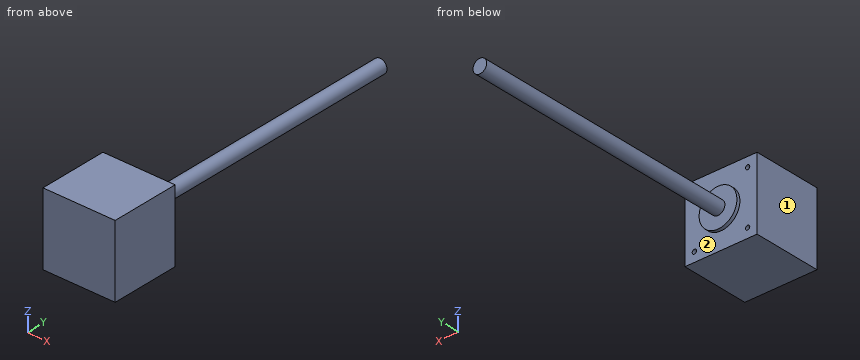
from build123d import *

# Parameters (mm, degrees)
SKETCH1_W             = 42
SKETCH1_H             = 42
BOSS_EXTRUDE1_DEPTH   = 40
SKETCH2_R             = 11
BOSS_EXTRUDE2_DEPTH   = 2
SKETCH3_R             = 4
BOSS_EXTRUDE3_DEPTH   = 159
SKETCH4_R             = 0.75
CUT_EXTRUDE1_DEPTH    = 5
M3_TAPPED_HOLE1_D     = 2.5
M3_TAPPED_HOLE1_DEPTH = 7.5
M3_TAPPED_HOLE1_TIP   = 0.751075774


with BuildPart() as part:
    # Sketch1 → Boss-Extrude1 (new body)
    with BuildSketch(Plane(origin=(0, 0, 0), x_dir=(1, 0, 0), z_dir=(0, 1, 0))):
        Rectangle(SKETCH1_W, SKETCH1_H)
    extrude(amount=BOSS_EXTRUDE1_DEPTH)

    # Sketch2 → Boss-Extrude2 (add)
    with BuildSketch(Plane(origin=(0, 40, 0), x_dir=(1, 0, 0), z_dir=(0, 1, 0))):
        with Locations(Location((0, 0, 0), (0, 0, 270))):
            Circle(SKETCH2_R)
    extrude(amount=BOSS_EXTRUDE2_DEPTH)

    # Sketch3 → Boss-Extrude3 (add)
    with BuildSketch(Plane(origin=(0, 42, 0), x_dir=(1, 0, 0), z_dir=(0, 1, 0))):
        with Locations(Location((0, 0, 0), (0, 0, 90))):
            Circle(SKETCH3_R)
    extrude(amount=BOSS_EXTRUDE3_DEPTH)

    # Sketch4 → Cut-Extrude1 (cut)
    with BuildSketch(Plane(origin=(0, 40, 0), x_dir=(1, 0, 0), z_dir=(0, 1, 0))):
        with Locations(Location((-15.5, 15.5, 0), (0, 0, 270))):
            Circle(SKETCH4_R)
        with Locations(Location((15.5, 15.5, 0), (0, 0, 270))):
            Circle(SKETCH4_R)
        with Locations(Location((15.5, -15.5, 0), (0, 0, 270))):
            Circle(SKETCH4_R)
        with Locations(Location((-15.5, -15.5, 0), (0, 0, 270))):
            Circle(SKETCH4_R)
    extrude(amount=-CUT_EXTRUDE1_DEPTH, mode=Mode.SUBTRACT)

    # M3 Tapped Hole1
    with Locations(Plane(origin=(0, 40, 0), x_dir=(1, 0, 0), z_dir=(0, 1, 0))):
        with Locations((-15.5, 15.5), (15.5, -15.5), (-15.5, -15.5), (15.5, 15.5)):
            Hole(M3_TAPPED_HOLE1_D / 2, depth=M3_TAPPED_HOLE1_DEPTH)
            with Locations((0, 0, -(M3_TAPPED_HOLE1_DEPTH + M3_TAPPED_HOLE1_TIP / 2))):  # 118° drill point
                Cone(0, M3_TAPPED_HOLE1_D / 2, M3_TAPPED_HOLE1_TIP, mode=Mode.SUBTRACT)


solid = part.part
Verification items for the finished model (mm, model axes). Face numbers are marked on the shaded views. A direction names the side the tool comes from. Give positions to 0.01 mm unless a question says otherwise; leave off trailing zeros. Write each loop counter-clockwise with the first axis right and the second up, starting at its lowest first coordinate (ties: lowest second). Pieces come first, ordered by that corner, then holes. Notation, with made-up numbers: (26, -18.75) - (59, -18.75) arc R16 cw to (59, -2.75) - close; hole circle Ø9 at (-32.5, -18.5). An arc over 180 degrees is marked (long way). Answer as CSV lines item,"result". Start each with the question number.
1. Sectioned sample at A-A (z = 0). Record the boundary of the cut face in (x, y), then the cut area to 3 significant figures.
2. Sectioned sample at B-B (x = 0). Record the boundary of the cut face in (y, z).
3. Set-up check for the marked faces 1 and 2: record each of +Z, -Z, +X, -X, +Y, -Y from which the full face is reachable in a straight line by a thin tool's end or side.
4. Thickness scan on line 1 (X direction, y = 35, z = -15.5); line 2 (X direction, y = 36, z = 15). Record the ranges inside material, lowest first.
5. Sectioned sample at C-C (y = 132). Record the boundary of the cut face in (x, z).
6. Depth check by flat-ended pin: pin 1 (12 mm diameter, centred on x = 1.5, y = 93, fed in from -Z); pin 2 (2 mm diameter, centred on y = 164, z = -5.5, fed in from +X); pin 3 (1 mm diameter, centred on y = 42, z = -2, fed in from +X); pin 4 (1.5 mm diameter, centred on x = 15.5, z = 15.5, fed in from +Y). Enter the tip coordinate at first touch or a pass-through.
Derived:
1,outline,"(-21, 0) - (21, 0) - (21, 40) - (11, 40) - (11, 42) - (4, 42) - (4, 201) - (-4, 201) - (-4, 42) - (-11, 42) - (-11, 40) - (-21, 40) - close"
1,area,"3,000 mm²"
2,outline,"(0, -21) - (40, -21) - (40, -11) - (42, -11) - (42, -4) - (201, -4) - (201, 4) - (42, 4) - (42, 11) - (40, 11) - (40, 21) - (0, 21) - close"
3,face 1,"+Z, -Z, -X, +Y, -Y"
3,face 2,"+Y"
4,line 1,"-21 to -16.75, -14.25 to 14.25, 16.75 to 21"
4,line 2,"-21 to -16.65, -14.35 to 14.35, 16.65 to 21"
5,outline,"circle Ø8 at (0, 0)"
6,pin 1,"z = -4"
6,pin 2,"through"
6,pin 3,"x = 10.9"
6,pin 4,"y = 32.2"
